from build123d import *

# Parameters (mm, degrees)
SKETCH1_R           = 40
BOSS_EXTRUDE1_DEPTH = 25


with BuildPart() as part:
    # Sketch1 → Boss-Extrude1 (new body)
    with BuildSketch(Plane.XY):
        with BuildLine():
            Line((17.320508076, 100), (601, 100))
            Line((601, 100), (601, 112))
            ThreePointArc((601, 112), (560.305386081, 134.762632261), (542.936006728, 178.034952402))
            ThreePointArc((542.936006728, 178.034952402), (518.682115493, 228.948270242), (465.174941276, 246.763979062))
            ThreePointArc((465.174941276, 246.763979062), (209.331516914, 209.226035995), (-39.530360121, 138.99270262))
            ThreePointArc((-39.530360121, 138.99270262), (-234.732763539, -32.083318616), (-258.432243095, -290.558303887))
            ThreePointArc((-258.432243095, -290.558303887), (-207.948857392, -337.074148263), (-143.032705856, -314.75399415))
            Line((-143.032705856, -314.75399415), (47.3, -89.6))
            Line((47.3, -89.6), (45.380171882, -78.3))
            ThreePointArc((45.380171882, -78.3), (-84.25636808, -33.032021404), (-19.925830789, 88.279166667))
            ThreePointArc((-19.925830789, 88.279166667), (-6.003449851, 109.077698758), (17.320508076, 100))
        make_face()
        with Locations((-194.2, -271.5)):
            Circle(SKETCH1_R, mode=Mode.SUBTRACT)
        with Locations((471, 175)):
            Circle(SKETCH1_R, mode=Mode.SUBTRACT)
    extrude(amount=BOSS_EXTRUDE1_DEPTH)


solid = part.part
Design review of the part built by this model. Coordinates are the model's own, in mm. A direction names the side the tool comes from. Coordinates: 2 decimals unless noted, no trailing zeros. Loops run counter-clockwise (first coordinate to the right, second up) from the corner with the lowest first, then second, coordinate; pieces in that order, holes last.
Item 1: Add section D-D (y = 0). Write out the cut boundary in (x, z).
Completed:
outline: (-216.18, 0) - (-90.5, 0) - (-90.5, 25) - (-216.18, 25) - close
Item 2: Wall thickness on L1, parallel to Y at x = 471, z = 17.5; L2, parallel to X at y = -276, z = 17; L3, parallel to X at y = -252.5, z = 5.75: over which ranges is each line inside the solid? List them lowest first.
Completed:
L1: y = 100 to 135, 215 to 247
L2: x = -262.41 to -233.95, -154.45 to -110.27
L3: x = -267.45 to -229.4, -159 to -90.41
Item 3: Draft analysis for pull direction X (two halves, no side actions). For faces 1 (the flat face through (33, 107, 0)), 2 (the cylindrical face through (-233.025, -28.776, 12.325)), 3 (the cylindrical face through (560.75, 134.26, 12.32)), 4 (the cylindrical face through (-202.87, -310.55, 12.32)), state which applies: pulls with the +X half, pulls with the -X half, needs draft (parallel to the pull), parting line crosses it, or undercut.
Completed:
face 1: needs draft
face 2: pulls with the -X half
face 3: pulls with the +X half
face 4: undercut
Item 4: Add section B-B (z = 20.5). Write out the cut boundary in (x, y).
Completed:
outline: (-258.43, -290.56) arc R67 ccw to (-143.03, -314.75) - (47.3, -89.6) - (45.38, -78.3) arc R90.5 cw (long way) to (-19.93, 88.28) arc R20 cw to (17.32, 100) - (601, 100) - (601, 112) arc R70 cw to (542.94, 178.03) arc R72 ccw to (465.17, 246.76) arc R2000 ccw to (-39.53, 138.99) arc R350 ccw to start; hole circle Ø80 at (-194.2, -271.5); hole circle Ø80 at (471, 175)
Item 5: For faces 5 (the cylindrical face through (-208.93, -336.86, 12.32)), 6 (the cylindrical face through (-6.36, 108.96, 12.32)), list the 3-axis set-ups (+Z, -Z, +X, -X, +Y, -Y) from which the entire face can be reached by the end or side of a thin tool; tool diameter is ignored.
Completed:
face 5: +Z, -Z, -Y
face 6: +Z, -Z
Item 6: Clearance check with flat-ended pins moving along their axes: pin 1 (12.5 mm diameter, centred on x = 273, z = 11, fed in from -Y); pin 2 (1.5 mm diameter, centred on y = -18, z = 20, fed in from +X); pin 3 (1 mm diameter, centred on y = 97.5, z = 19, fed in from +X). State where each tip first meets the part, or that it passes through.
Completed:
pin 1: stops at y = 100
pin 2: stops at x = -88.54
pin 3: stops at x = -18.33
Item 7: Add section A-A (x = 0). Write out the cut boundary in (y, z), and give its area (3 significant figures).
Completed:
outline: (-145.55, 0) - (-90.5, 0) - (-90.5, 25) - (-145.55, 25) - close; (110, 0) - (152.5, 0) - (152.5, 25) - (110, 25) - close
area: 2,440 mm2
Item 8: Add section C-C (y = -271.5). Write out the cut boundary in (x, z).
Completed:
outline: (-263.51, 0) - (-234.2, 0) - (-234.2, 25) - (-263.51, 25) - close; (-154.2, 0) - (-106.47, 0) - (-106.47, 25) - (-154.2, 25) - close
